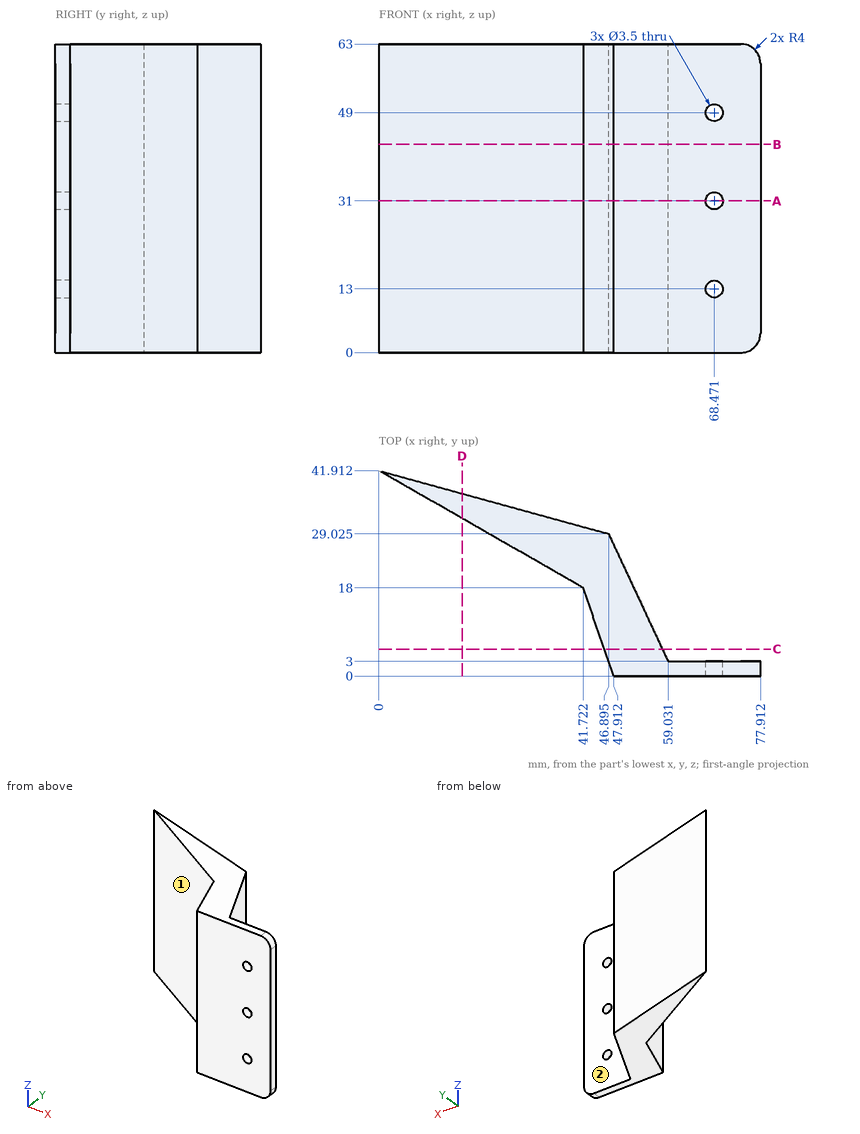
Check sheet for the drawn part. Datum: minimum x, y, z corner. Units: mm. A direction names the side the tool comes from. Round coordinates to 2 decimals unless told otherwise and drop trailing zeros. Loops run counter-clockwise (first coordinate to the right, second up) from the corner with the lowest first, then second, coordinate; pieces in that order, holes last. Notation, with made-up numbers: (82, 54.25) -> (128, 54.25) arc R16 cw to (128, 85.25) -> close; hole circle Ø10 at (-22, -38.5). An arc over 180 degrees is marked (long way). Put each result on its own line as item: value. Start each with the question number.
1. Scan lines: probe 1 along Y at (x, z) = (70.5, 14); probe 2 along X at (y, z) = (1.2, 49); probe 3 along X at (y, z) = (2, 31) (1 decimal). Record each from-to range of solid material in increasing order.
2. Section check C-C (y = 5.5). Enter the section's corners in (x, z) (1 decimal), plus the area to 3 significant figures.
3. Gauge pin test, flat ends, axial feed: pin 1 (6 mm diameter, centred on x = 10.5, z = 9, fed in from +Y); pin 2 (4 mm diameter, centred on x = 68.47, z = 49, fed in from +Y); pin 3 (6 mm diameter, centred on x = 35.5, z = 37, fed in from +Y). Record the tip position at first contact, or that the pin passes through.
4. Section check D-D (x = 17). Enter the section's corners in (y, z).
5. Section check A-A (z = 31). Enter the section's corners in (x, y) (1 decimal), plus the area to 3 significant figures.
6. Section check B-B (z = 42.5). Enter the section's corners in (x, y) (1 decimal), plus the area to 3 significant figures.
7. Access from +Z, -Z, +X, -X, +Y, -Y to the whole of each face (thin tool, end or side, straight path). Record for the marked faces 1 and 2.
Findings:
1. probe 1: y = 0 to 3
1. probe 2: x = 47.5 to 66.72, 70.22 to 77.91
1. probe 3: x = 47.2 to 66.7, 70.2 to 77.9
2. outline: (46, 0) -> (57.9, 0) -> (57.9, 63) -> (46, 63) -> close
2. area: 746 mm^2
3. pin 1: stops at y = 39.85
3. pin 2: stops at y = 3
3. pin 3: stops at y = 32.98
4. outline: (32.17, 0) -> (37.24, 0) -> (37.24, 63) -> (32.17, 63) -> close
5. outline: (0, 41.9) -> (41.7, 18) -> (47.9, 0) -> (66.7, 0) -> (66.7, 3) -> (59, 3) -> (46.9, 29) -> close; (70.2, 0) -> (77.9, 0) -> (77.9, 3) -> (70.2, 3) -> close
5. area: 598 mm^2
6. outline: (0, 41.9) -> (41.7, 18) -> (47.9, 0) -> (77.9, 0) -> (77.9, 3) -> (59, 3) -> (46.9, 29) -> close
6. area: 609 mm^2
7. face 1: +Z, -Z, -X, -Y
7. face 2: +Z, -Z, +X, +Y
